For this review, take the finished solid that the model builds, in its own axes (mm). A direction names the side the tool comes from. Round coordinates to 2 decimals unless told otherwise and drop trailing zeros. Order: outer loops, then holes, each group sorted by start corner. A loop starts at its lowest first (then second) coordinate and runs counter-clockwise, first axis right, second up. Notation, with made-up numbers: M 44,-34.75 L 60,-34.75 A15 ccw 60,-18.75 Z; hole C -23,52.25 d4. An arc over 180 degrees is marked long. Put each result on its own line as item: value.
from build123d import *

# Parameters (mm, degrees)
SKETCH1_R           = 5
BOSS_EXTRUDE1_DEPTH = 2
SKETCH2_R           = 3
BOSS_EXTRUDE2_DEPTH = 14
CHAMFER1_SIZE       = 0.5


with BuildPart() as part:
    # Sketch1 → Boss-Extrude1 (new body)
    with BuildSketch(Plane(origin=(0, 0, 0), x_dir=(1, 0, 0), z_dir=(0, 1, 0))):
        with Locations(Location((0, 0, 0), (0, 0, 270))):
            Circle(SKETCH1_R)
    extrude(amount=BOSS_EXTRUDE1_DEPTH)

    # Sketch2 → Boss-Extrude2 (add)
    with BuildSketch(Plane(origin=(0, 2, 0), x_dir=(1, 0, 0), z_dir=(0, 1, 0))):
        with Locations(Location((0, 0, 0), (0, 0, 270))):
            Circle(SKETCH2_R)
    extrude(amount=BOSS_EXTRUDE2_DEPTH)

    # Chamfer1
    chamfer1_edges = [part.edges().sort_by_distance(p)[0] for p in [
        (0, 0, -5),
        (0, 16, -3),
    ]]
    chamfer(chamfer1_edges, length=CHAMFER1_SIZE)


solid = part.part
(1) Insertion check: pin 1 Ø2 at (y, z) = (11.5, 1) entering from -X; pin 2 Ø2 at (x, y) = (-2.5, 13) entering from +Z; pin 3 Ø4 at (x, y) = (3, 12.5) entering from +Z; pin 4 Ø1.5 at (x, z) = (-3.5, 0) entering from -Y. Each pin has a flat end and moves straight along its axis. Give the tip position at first contact, or say it passes through.
A:
pin 1: stops at x = -3
pin 2: stops at z = 2.6
pin 3: stops at z = 2.83
pin 4: stops at y = 0
(2) Add section B-B on y = 9.25. Give the boundary of the cut face in (x, z).
A:
outline: C 0,0 d6
(3) For faces 1 (the face through (0, 16, 0)), 2 (the face through (-3.3, 2, -0.1)), list the 3-axis set-ups (+Z, -Z, +X, -X, +Y, -Y) from which the entire face can be reached by the end or side of a thin tool; tool diameter is ignored.
A:
face 1: +Z, -Z, +X, -X, +Y
face 2: +Y
(4) Add section A-A on z = 0. Give the boundary of the cut face in (x, y), then the cut area to 4 significant figures.
A:
outline: M -5,0.5 L -4.5,0 L 4.5,0 L 5,0.5 L 5,2 L 3,2 L 3,15.5 L 2.5,16 L -2.5,16 L -3,15.5 L -3,2 L -5,2 Z
area: 103.5 mm2
(5) To check wall thickness, follow L1, parallel to Y at x = -3.75, z = -1.5; L2, parallel to X at y = 12.75, z = 2; L3, parallel to X at y = 1.5, z = -0.5. State the ranges of each line that lie inside material, in increasing order.
A:
L1: y = 0 to 2
L2: x = -2.24 to 2.24
L3: x = -4.97 to 4.97
